Can you work these out from the drawing? Everything is in mm from the part's minimum corner. A direction names the side the tool comes from. Give positions to 0.01 mm unless a question says otherwise; leave off trailing zeros. Loops run counter-clockwise (first coordinate to the right, second up) from the corner with the lowest first, then second, coordinate; pieces in that order, holes last.
Q1. For the marked faces 4, 5 and 6, which set-ups out of +Z, -Z, +X, -X, +Y, -Y let a thin tool reach every point of the face, with its end or its side?
Q2. I need wall thicknesses on line 1 (X direction, y = 55, z = 43); line 2 (Y direction, x = 23, z = 43); line 3 (Y direction, x = 7, z = 7). Which ranges of each line are inside material? Lowest first, please.
Q3. Will these pins go through, and if not, where does the flat tip stop? P1, Ø4, axis at x = 13.5, y = 35, coming from the -Z side; P2, Ø10, axis at x = 32.5, y = 40, coming from the +Z side; P3, Ø2, axis at y = 66, z = 42.5, coming from the +X side; P4, Ø10, axis at y = 9, z = 11.5, coming from the -X side.
Q4. We'd pull the mould along X, two halves only. Please class the marked faces 1, 2 and 3: +X half, -X half, draft (parallel to the pull), parting line (faces both ways), or undercut.
Q5. If we section it at B-B (z = 57.5): Please give me the cut outline in (x, y), plus the area to 3 significant figures.
Q6. If we section it at A-A (x = 23): Please give me the cut outline in (y, z).
Q7. If we section it at D-D (y = 57): Please give me the cut outline in (x, z), plus the area to 3 significant figures.
Q8. If we section it at C-C (y = 25): Please give me the cut outline in (x, z), plus the area to 3 significant figures.
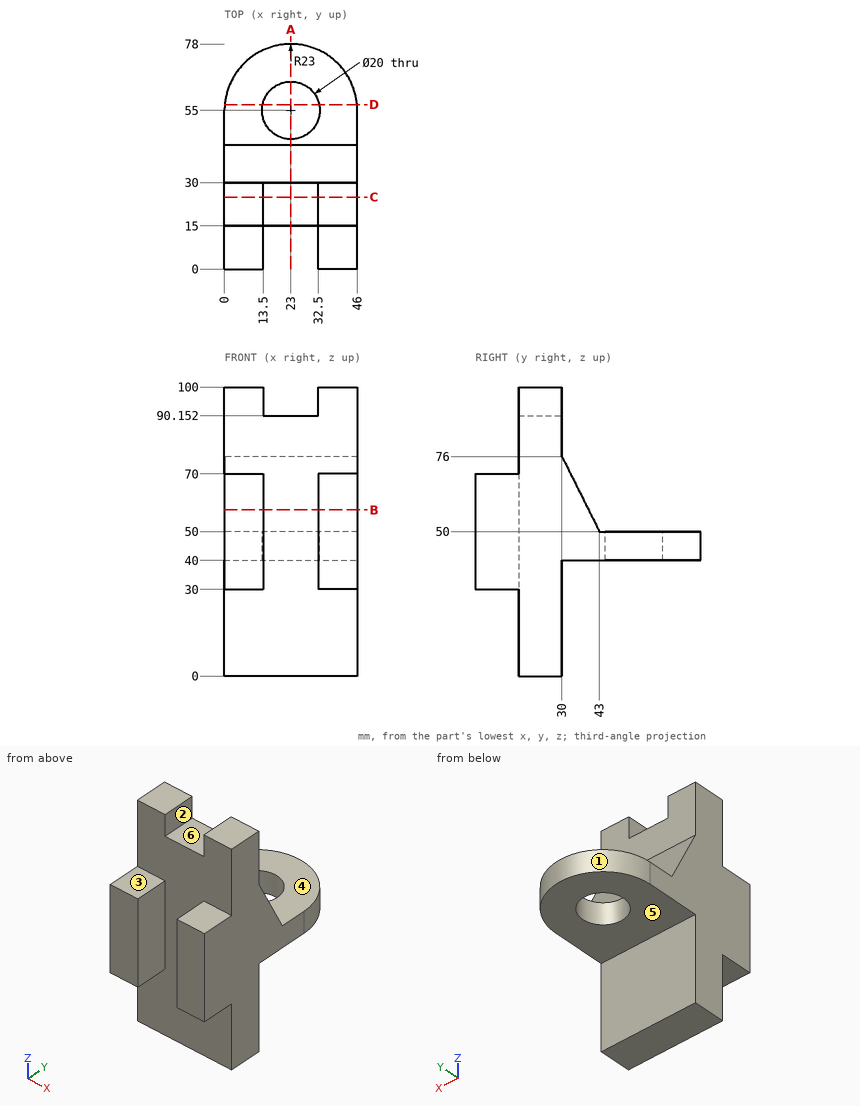
Check sheet entries:
1. face 4: +Z, +X, -X, +Y
1. face 5: -Z, +X, -X, +Y
1. face 6: +Z, +Y, -Y
2. line 1: x = 0 to 13, 33 to 46
2. line 2: y = 15 to 45, 65 to 78
2. line 3: y = 15 to 30
3. P1: stops at z = 40
3. P2: stops at z = 66
3. P3: stops at x = 43.71
3. P4: passes through
4. face 1: parting line
4. face 2: undercut
4. face 3: draft
5. outline: (0, 0) - (13.5, 0) - (13.5, 15) - (32.5, 15) - (32.5, 0) - (46, 0) - (46, 39.25) - (0, 39.25) - close
5. area: 1,520 mm2
6. outline: (15, 0) - (30, 0) - (30, 40) - (45, 40) - (45, 50) - (43, 50) - (30, 76) - (30, 90.15) - (15, 90.15) - close; (65, 40) - (78, 40) - (78, 50) - (65, 50) - close
7. outline: (0.09, 40) - (13.2, 40) - (13.2, 50) - (0.09, 50) - close; (32.8, 40) - (45.91, 40) - (45.91, 50) - (32.8, 50) - close
7. area: 262 mm2
8. outline: (0, 0) - (46, 0) - (46, 100) - (32.5, 100) - (32.5, 90.15) - (13.5, 90.15) - (13.5, 100) - (0, 100) - close
8. area: 4,410 mm2
